Input: dimensioned drawing with shaded views. Units: mm. Origin: part minimum x, y, z. Round coordinates to 2 decimals unless told otherwise and drop trailing zeros. Loops run counter-clockwise (first coordinate to the right, second up) from the corner with the lowest first, then second, coordinate; pieces in that order, holes last.
Item 1: Ray query, L1, parallel to Y at x = 13, z = 0.6; L2, parallel to Y at x = 53, z = 1.05; L3, parallel to Y at x = 71, z = 1.75. Return the intervals inside material, ascending.
Item 2: Section query B-B on x = 71. Return loops of the section in (y, z).
Item 3: Section query A-A on y = 53. Return loops of the section in (x, z), then the cut area to 3 significant figures.
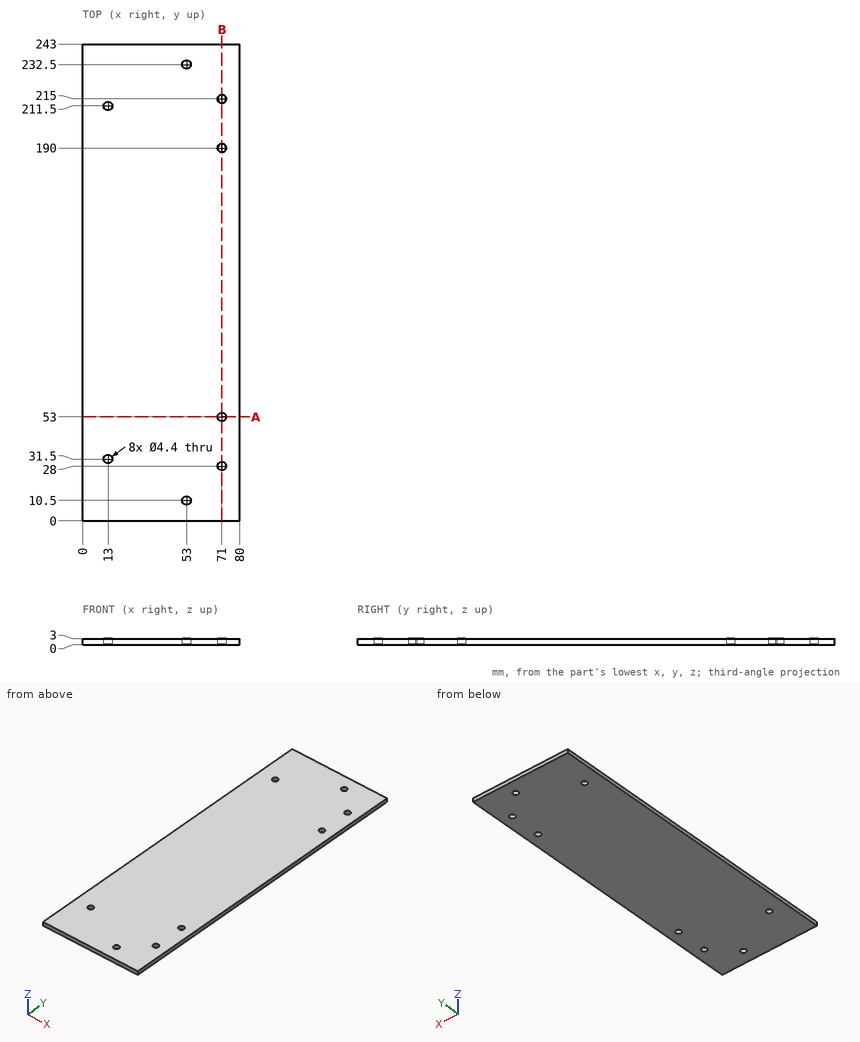
Data:
1. L1: y = 0 to 29.3, 33.7 to 209.3, 213.7 to 243
1. L2: y = 0 to 8.3, 12.7 to 230.3, 234.7 to 243
1. L3: y = 0 to 25.8, 30.2 to 50.8, 55.2 to 187.8, 192.2 to 212.8, 217.2 to 243
2. outline: (0, 0) - (25.8, 0) - (25.8, 3) - (0, 3) - close; (30.2, 0) - (50.8, 0) - (50.8, 3) - (30.2, 3) - close; (55.2, 0) - (187.8, 0) - (187.8, 3) - (55.2, 3) - close; (192.2, 0) - (212.8, 0) - (212.8, 3) - (192.2, 3) - close; (217.2, 0) - (243, 0) - (243, 3) - (217.2, 3) - close
3. outline: (0, 0) - (68.8, 0) - (68.8, 3) - (0, 3) - close; (73.2, 0) - (80, 0) - (80, 3) - (73.2, 3) - close
3. area: 227 mm2
